from build123d import *

# Parameters (mm, degrees)
SKETCH1_R           = 8
SKETCH1_R_2         = 2.25
BOSS_EXTRUDE1_DEPTH = 1.5
SKETCH2_OUTSIDE_W   = 22.566
SKETCH2_OUTSIDE_H   = 22.566
SKETCH2_OUTSIDE_W_2 = 20
SKETCH2_OUTSIDE_H_2 = 10
CUT_EXTRUDE1_DEPTH  = 12.704699911
CHAMFER1_SIZE       = 0.3


with BuildPart() as part:
    # Sketch1 → Boss-Extrude1 (new, symmetric)
    with BuildSketch(Plane.XY):
        Circle(SKETCH1_R)
        Circle(SKETCH1_R_2, mode=Mode.SUBTRACT)
    extrude(amount=BOSS_EXTRUDE1_DEPTH, both=True)

    # Sketch2 outside → Cut-Extrude1 (cut, through all)
    with BuildSketch(Plane.XY.offset(1.5)):
        Rectangle(SKETCH2_OUTSIDE_W, SKETCH2_OUTSIDE_H)
        Rectangle(SKETCH2_OUTSIDE_W_2, SKETCH2_OUTSIDE_H_2, mode=Mode.SUBTRACT)
    extrude(amount=-CUT_EXTRUDE1_DEPTH, mode=Mode.SUBTRACT)

    # Chamfer1
    chamfer1_edges = [part.edges().sort_by_distance(p)[0] for p in [
        (8, 0, 1.5),
        (-8, 0, -1.5),
        (8, 0, -1.5),
        (0, 5, -1.5),
        (0, -5, -1.5),
        (0, -5, 1.5),
        (0, 5, 1.5),
        (-2.25, 0, -1.5),
        (-2.25, 0, 1.5),
        (-8, 0, 1.5),
    ]]
    chamfer(chamfer1_edges, length=CHAMFER1_SIZE)


solid = part.part
Build history of the part. All positions in model axes, mm. Round coordinates to 2 decimals unless told otherwise and drop trailing zeros. Write each loop counter-clockwise with the first axis right and the second up, starting at its lowest first coordinate (ties: lowest second). Pieces come first, ordered by that corner, then holes. Notation, with made-up numbers: (35, -33) -> (86, -33) arc R17 cw to (86, -2) -> close; hole circle Ø8 at (-32.75, 5.25). An arc over 180 degrees is marked (long way). Use one line per item in the form item = value.
Q1. Drop flat-ended pins along their axis: P1, Ø1.5, axis at y = 3, z = 1, coming from the +X side; P2, Ø1.5, axis at y = 3.5, z = -0.5, coming from the -X side; P3, Ø2.5, axis at x = 0, y = 0, coming from the +Z side. Give the stop position or say it passes through.
Conclusion:
P1 = 7.68
P2 = -7.51
P3 = through
Q2. Band-saw the part on B-B, the plane y = 0. Write the cut outline in (x, z), then the cut area to 3 significant figures.
Conclusion:
outline = (-8, -1.2) -> (-7.7, -1.5) -> (-2.55, -1.5) -> (-2.25, -1.2) -> (-2.25, 1.2) -> (-2.55, 1.5) -> (-7.7, 1.5) -> (-8, 1.2) -> close; (2.25, -1.2) -> (2.55, -1.5) -> (7.7, -1.5) -> (8, -1.2) -> (8, 1.2) -> (7.7, 1.5) -> (2.55, 1.5) -> (2.25, 1.2) -> close
area = 34.1 mm²
Q3. Drill centre lines: L1, parallel to Y at x = 0, z = 0.6; L2, parallel to X at y = -1, z = -0.3; L3, parallel to X at y = 1.5, z = -1.3. Where is each one in solid material? Low to high.
Conclusion:
L1 = -5 to -2.25, 2.25 to 5
L2 = -7.94 to -2.02, 2.02 to 7.94
L3 = -7.76 to -1.81, 1.81 to 7.76
Q4. Band-saw the part on A-A, the plane x = 0. Write the cut outline in (y, z), then the cut area to 3 significant figures.
Conclusion:
outline = (-5, -1.2) -> (-4.7, -1.5) -> (-2.55, -1.5) -> (-2.25, -1.2) -> (-2.25, 1.2) -> (-2.55, 1.5) -> (-4.7, 1.5) -> (-5, 1.2) -> close; (2.25, -1.2) -> (2.55, -1.5) -> (4.7, -1.5) -> (5, -1.2) -> (5, 1.2) -> (4.7, 1.5) -> (2.55, 1.5) -> (2.25, 1.2) -> close
area = 16.1 mm²
Q5. Two-plate mould, pull along Y, no slides. Class faces 1 (the cylindrical face through (-0.29, 2.23, -0.02)), 2 (the conical face through (7.81, -0.07, -1.39)), 3 (the flat face through (-2, -2, 1.5)), 4 (the flat face through (0, -5, 0)): released by +Y, released by -Y, zero draft, split by the parting line, or undercut.
Conclusion:
face_1 = undercut
face_2 = split by the parting line
face_3 = zero draft
face_4 = released by -Y
Q6. Band-saw the part on C-C, the plane z = 0.5. Write the cut outline in (x, y) (3 decimals), then the cut area to 3 significant figures.
Conclusion:
outline = (-6.245, -5) -> (6.245, -5) arc R8 ccw to (6.245, 5) -> (-6.245, 5) arc R8 ccw to start; hole circle Ø4.5 at (0, 0)
area = 133 mm²
